Design review of the part built by this model. Coordinates are the model's own, in mm. Face numbers are marked on the shaded views. Coordinates: 2 decimals unless noted, no trailing zeros. Loops run counter-clockwise (first coordinate to the right, second up) from the corner with the lowest first, then second, coordinate; pieces in that order, holes last.
Q1. Add section A-A on z = -55. Give the boundary of the cut face in (x, y).
Q2. Add section C-C on z = 60. Give the boundary of the cut face in (x, y), and give its area (3 significant figures).
Q3. For P1, Ø12, axis at x = -39.5, z = 24.5, coming from the -Y side; P2, Ø10, axis at x = -155, z = 75, coming from the +Y side (3 decimals); P3, Ø8, axis at x = -28, z = 60, coming from the +Y side; P4, Ø7, axis at x = -23, z = -105, coming from the +Y side, all flat-tipped, find the tip position at first contact; note any pin that passes through.
Q4. Wall thickness on probe 1 along X at (y, z) = (14, -55); probe 2 along X at (y, z) = (24, 20); probe 3 along X at (y, z) = (7, 60): over which ranges is each line inside the solid? List them lowest first.
Q5. Add section B-B on y = 26.5. Give the number of separate pieces and of enclosed holes in the cut face, and give its area (3 significant figures).
Q6. Draft analysis for pull direction Z (two halves, no side actions). For the marked faces 1, 2 and 3, state which applies: released by +Z, released by -Z, zero draft, split by the parting line, or undercut.
```python
from build123d import *

# Parameters (mm, degrees)
SKETCH1_R                    = 20
SKETCH1_R_2                  = 4.5
BOSS_EXTRUDE1_DEPTH          = 40
SKETCH2_R                    = 7
CUT_EXTRUDE1_DEPTH           = 9
M10_TAPPED_HOLE1_D           = 8.5
M10_TAPPED_HOLE1_DEPTH       = 27.5
M10_TAPPED_HOLE1_CSINK_D     = 10.05
M10_TAPPED_HOLE1_CSINK_ANGLE = 90
M10_TAPPED_HOLE1_TIP         = 2.553657631


with BuildPart() as part:
    # Sketch1 → Boss-Extrude1 (new body)
    with BuildSketch(Plane(origin=(0, 0, 0), x_dir=(1, 0, 0), z_dir=(0, 1, 0))):
        with BuildLine():
            Line((-170, -125), (170, -125))
            ThreePointArc((170, -125), (177.071067812, -122.071067812), (180, -115))
            Line((180, -115), (180, 115))
            ThreePointArc((180, 115), (177.071067812, 122.071067812), (170, 125))
            Line((170, 125), (-170, 125))
            ThreePointArc((-170, 125), (-177.071067812, 122.071067812), (-180, 115))
            Line((-180, 115), (-180, -115))
            ThreePointArc((-180, -115), (-177.071067812, -122.071067812), (-170, -125))
        make_face()
        with Locations(Location((-110, 55, 0), (0, 0, 270))):
            Circle(SKETCH1_R, mode=Mode.SUBTRACT)
        with Locations(Location((110, 55, 0), (0, 0, 270))):
            Circle(SKETCH1_R, mode=Mode.SUBTRACT)
        with Locations(Location((0, -85, 0), (0, 0, 270))):
            Circle(SKETCH1_R_2, mode=Mode.SUBTRACT)
        with Locations(Location((0, -30, 0), (0, 0, 270))):
            Circle(SKETCH1_R_2, mode=Mode.SUBTRACT)
        with Locations(Location((28, -60, 0), (0, 0, 270))):
            Circle(SKETCH1_R_2, mode=Mode.SUBTRACT)
        with Locations(Location((-28, -60, 0), (0, 0, 270))):
            Circle(SKETCH1_R_2, mode=Mode.SUBTRACT)
    extrude(amount=BOSS_EXTRUDE1_DEPTH)

    # Sketch2 → Cut-Extrude1 (cut)
    with BuildSketch(Plane.XZ):
        with Locations(Location((0, 30, 0), (0, 0, 270))):
            Circle(SKETCH2_R)
        with Locations(Location((-28, 60, 0), (0, 0, 270))):
            Circle(SKETCH2_R)
        with Locations(Location((0, 85, 0), (0, 0, 270))):
            Circle(SKETCH2_R)
        with Locations(Location((28, 60, 0), (0, 0, 270))):
            Circle(SKETCH2_R)
    extrude(amount=-CUT_EXTRUDE1_DEPTH, mode=Mode.SUBTRACT)

    # M10 Tapped Hole1
    with Locations(Plane(origin=(0, 40, 0), x_dir=(1, 0, 0), z_dir=(0, 1, 0))):
        with Locations((-23, 105), (-155, -35), (-155, -75), (-107.5, -20), (-67.5, -20), (-107.5, -90), (-67.5, -90), (155, -75), (155, -35), (67.5, -90), (107.5, -90), (67.5, -20), (107.5, -20), (23, 105)):
            CounterSinkHole(M10_TAPPED_HOLE1_D / 2, M10_TAPPED_HOLE1_CSINK_D / 2, depth=M10_TAPPED_HOLE1_DEPTH, counter_sink_angle=M10_TAPPED_HOLE1_CSINK_ANGLE)
            with Locations((0, 0, -(M10_TAPPED_HOLE1_DEPTH + M10_TAPPED_HOLE1_TIP / 2))):  # 118° drill point
                Cone(0, M10_TAPPED_HOLE1_D / 2, M10_TAPPED_HOLE1_TIP, mode=Mode.SUBTRACT)


solid = part.part
```
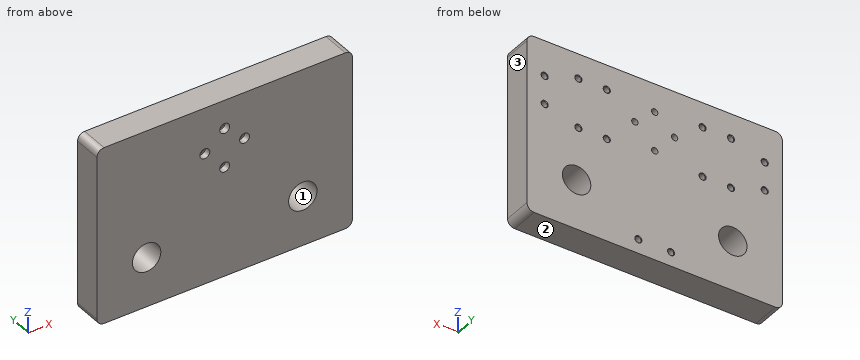
Entries:
1. outline: (-180, 0) - (-130, 0) - (-130, 40) - (-180, 40) - close; (-90, 0) - (90, 0) - (90, 40) - (-90, 40) - close; (130, 0) - (180, 0) - (180, 40) - (130, 40) - close
2. outline: (-180, 0) - (-35, 0) - (-35, 9) - (-32.5, 9) - (-32.5, 40) - (-180, 40) - close; (-23.5, 9) - (-21, 9) - (-21, 0) - (21, 0) - (21, 9) - (23.5, 9) - (23.5, 40) - (-23.5, 40) - close; (32.5, 9) - (35, 9) - (35, 0) - (180, 0) - (180, 40) - (32.5, 40) - close
2. area: 13,600 mm2
3. P1: stops at y = 0
3. P2: stops at y = 39.975
3. P3: passes through
3. P4: stops at y = 12.05
4. probe 1: x = -180 to -130, -90 to 90, 130 to 180
4. probe 2: x = -180 to -111.75, -103.25 to -71.75, -63.25 to 63.25, 71.75 to 103.25, 111.75 to 180
4. probe 3: x = -180 to -35, -21 to 21, 35 to 180
5. separate pieces: 1
5. enclosed holes: 20
5. area: 86,400 mm2
6. face 1: undercut
6. face 2: released by -Z
6. face 3: zero draft
